```python
from build123d import *

# Parameters (mm, degrees)
BOSS_EXTRUDE1_DEPTH = 14
SKETCH3_R           = 11.5
CUT_EXTRUDE1_DEPTH  = 14
SKETCH4_R           = 10
BOSS_EXTRUDE2_DEPTH = 20


with BuildPart() as part:
    # Sketch2 → Boss-Extrude1 (new body)
    with BuildSketch(Plane(origin=(0, 0, 0), x_dir=(1, 0, 0), z_dir=(0, 1, 0))):
        Polygon((0, 0), (0, 120), (60, 120), (120, 60), (120, 0), align=None)
    extrude(amount=BOSS_EXTRUDE1_DEPTH)

    # Sketch3 → Cut-Extrude1 (cut)
    with BuildSketch(Plane(origin=(0, 14, 0), x_dir=(1, 0, 0), z_dir=(0, 1, 0))):
        with Locations(Location((40, 40, 0), (0, 0, 270))):
            Circle(SKETCH3_R)
    extrude(amount=-CUT_EXTRUDE1_DEPTH, mode=Mode.SUBTRACT)

    # Sketch4 → Boss-Extrude2 (add)
    with BuildSketch(Plane(origin=(0, 14, 0), x_dir=(1, 0, 0), z_dir=(0, 1, 0))):
        Polygon((57.320508076, 40), (48.660254038, 55), (31.339745962, 55), (22.679491924, 40), (31.339745962, 25), (48.660254038, 25), align=None)
        with Locations(Location((40, 40, 0), (0, 0, 270))):
            Circle(SKETCH4_R, mode=Mode.SUBTRACT)
    extrude(amount=BOSS_EXTRUDE2_DEPTH)


solid = part.part
```
Design review of the part built by this model. Coordinates are the model's own, in mm. A direction names the side the tool comes from. Coordinates: 2 decimals unless noted, no trailing zeros. Order: outer loops, then holes, each group sorted by start corner. A loop starts at its lowest first (then second) coordinate and runs counter-clockwise, first axis right, second up. Notation, with made-up numbers: M -20.75,86 L -9.75,86 A27 ccw -9.75,116 Z; hole C -14,42 d2. An arc over 180 degrees is marked long. Answer as a JSON object with one key per item and string values. Group by question number.
1) Add section A-A, the plane x = 40. Write out the cut boundary in (y, z).
2) For pin 1 (6 mm diameter, centred on x = 102.5, z = -15, fed in from +Y); pin 2 (20.5 mm diameter, centred on x = 40, z = -40, fed in from -Y); pin 3 (6 mm diameter, centred on x = 83, y = 11, fed in from -Z); pin 4 (16 mm diameter, centred on x = 40, z = -40, fed in from +Y) (3 decimals), all flat-tipped, find the tip position at first contact; note any pin that passes through.
3) Add section C-C, the plane z = -34.5. Write out the cut boundary in (x, y), then the cut area to 3 significant figures.
4) Mouldability with a two-part tool opening along X and no side actions: class faces 1 (the flat face through (120, 7, -30)), 2 (the flat face through (27.07, 23.86, -47.605)), 3 (the cylindrical face through (30.24, 23.86, -42.17)), 4 (the flat face through (61, 0, -61)) as pulls with the +X half, pulls with the -X half, needs draft (parallel to the pull), parting line crosses it, or undercut.
5) Add section D-D, the plane z = -94. Write out the cut boundary in (x, y), then the cut area to 3 significant figures.
6) Tool access review of faces 5 (the flat face through (40, 24, -25)), 6 (the flat face through (26.95, 23.86, -32.6)), 7 (the flat face through (40, 24, -55)), 8 (the flat face through (52.93, 23.86, -32.395)): name each direction out of +Z, -Z, +X, -X, +Y, -Y from which nothing blocks a thin tool from reaching the whole face with its end or side.
7) Add section B-B, the plane y = 18. Write out the cut boundary in (x, z), then the cut area to 3 significant figures.
8) Wall thickness on L1, parallel to X at y = 7.75, z = -40; L2, parallel to Y at x = 88, z = -54.5; L3, parallel to Z at x = 49, y = 4: over which ranges is each line inside the solid? List them lowest first.
Computed values:
{
 "1": {"outline": "M 0,-120 L 14,-120 L 14,-55 L 34,-55 L 34,-50 L 14,-50 L 14,-51.5 L 0,-51.5 Z; M 0,-28.5 L 14,-28.5 L 14,-30 L 34,-30 L 34,-25 L 14,-25 L 14,0 L 0,0 Z"},
 "2": {"pin 1": "stops at y = 14", "pin 2": "stops at y = 14", "pin 3": "stops at z = -100", "pin 4": "passes through"},
 "3": {"outline": "M 0,0 L 29.9,0 L 29.9,14 L 31.65,14 L 31.65,34 L 25.85,34 L 25.85,14 L 0,14 Z; M 48.35,14 L 50.1,14 L 50.1,0 L 120,0 L 120,14 L 54.15,14 L 54.15,34 L 48.35,34 Z", "area": "1,630 mm^2"},
 "4": {"face 1": "pulls with the +X half", "face 2": "pulls with the -X half", "face 3": "undercut", "face 4": "needs draft"},
 "5": {"outline": "M 0,0 L 86,0 L 86,14 L 0,14 Z", "area": "1,200 mm^2"},
 "6": {"face 5": "+Z, +X, -X, +Y", "face 6": "+Z, -X, +Y", "face 7": "-Z, +X, -X, +Y", "face 8": "+Z, +X, +Y"},
 "7": {"outline": "M 22.68,-40 L 31.34,-55 L 48.66,-55 L 57.32,-40 L 48.66,-25 L 31.34,-25 Z; hole C 40,-40 d20", "area": "465 mm^2"},
 "8": {"L1": "x = 0 to 28.5, 51.5 to 120", "L2": "y = 0 to 14", "L3": "z = -120 to -47.16, -32.84 to 0"}
}
